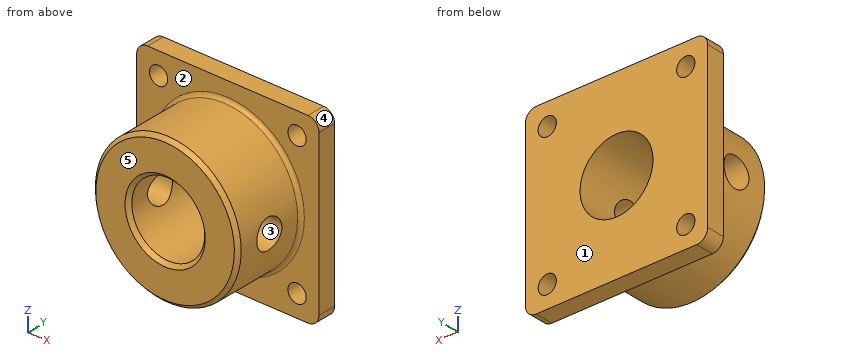
from build123d import *

# Parameters (mm, degrees)
SKETCH1_R               = 20
BOSS_EXTRUDE1_DEPTH     = 20
CUT_EXTRUDE5_DEPTH      = 25
CUT_EXTRUDE5_DEPTH_BACK = 25
SKETCH8_R               = 4
SKETCH9_W               = 50
SKETCH9_H               = 50
BOSS_EXTRUDE3_DEPTH     = 5
SKETCH10_R              = 10
CUT_EXTRUDE6_DEPTH      = 25
SKETCH11_R              = 2.5
CUT_EXTRUDE7_DEPTH      = 10
FILLET1_R               = 3
FILLET2_R               = 1
CHAMFER1_SIZE           = 1


with BuildPart() as part:
    # Sketch1 → Boss-Extrude1 (new body)
    with BuildSketch(Plane(origin=(0, 0, 0), x_dir=(1, 0, 0), z_dir=(0, 1, 0))):
        with Locations(Location((0, 0, 0), (0, 0, 270))):
            Circle(SKETCH1_R)
    extrude(amount=BOSS_EXTRUDE1_DEPTH)

    # Sketch8 → Cut-Extrude5 (cut, two sides: drawn at the far end of the back side and taken through both)
    with BuildSketch(Plane(origin=(0, 0, 0), x_dir=(0, 0, -1), z_dir=(1, 0, 0)).offset(-CUT_EXTRUDE5_DEPTH_BACK)):
        with Locations(Location((0, 10, 0), (0, 0, 180))):
            Circle(SKETCH8_R)
    extrude(amount=CUT_EXTRUDE5_DEPTH + CUT_EXTRUDE5_DEPTH_BACK, mode=Mode.SUBTRACT)

    # Sketch9 → Boss-Extrude3 (add)
    with BuildSketch(Plane(origin=(0, 20, 0), x_dir=(1, 0, 0), z_dir=(0, 1, 0))):
        Rectangle(SKETCH9_W, SKETCH9_H)
    extrude(amount=BOSS_EXTRUDE3_DEPTH)

    # Sketch10 → Cut-Extrude6 (cut)
    with BuildSketch(Plane(origin=(0, 25, 0), x_dir=(1, 0, 0), z_dir=(0, 1, 0))):
        with Locations(Location((0, 0, 0), (0, 0, 270))):
            Circle(SKETCH10_R)
    extrude(amount=-CUT_EXTRUDE6_DEPTH, mode=Mode.SUBTRACT)

    # Sketch11 → Cut-Extrude7 (cut)
    with BuildSketch(Plane(origin=(0, 25, 0), x_dir=(1, 0, 0), z_dir=(0, 1, 0))):
        with Locations(Location((-19, 19, 0), (0, 0, 270))):
            Circle(SKETCH11_R)
        with Locations(Location((-19, -19, 0), (0, 0, 270))):
            Circle(SKETCH11_R)
        with Locations(Location((19, -19, 0), (0, 0, 270))):
            Circle(SKETCH11_R)
        with Locations(Location((19, 19, 0), (0, 0, 270))):
            Circle(SKETCH11_R)
    extrude(amount=-CUT_EXTRUDE7_DEPTH, mode=Mode.SUBTRACT)

    # Fillet1
    fillet1_edges = [part.edges().sort_by_distance(p)[0] for p in [
        (25, 22.5, 25),
        (25, 22.5, -25),
        (-25, 22.5, -25),
        (-25, 22.5, 25),
    ]]
    fillet(fillet1_edges, radius=FILLET1_R)

    # Fillet2
    fillet2_edges = [part.edges().sort_by_distance(p)[0] for p in [
        (0, 20, -20),
    ]]
    fillet(fillet2_edges, radius=FILLET2_R)

    # Chamfer1
    chamfer1_edges = [part.edges().sort_by_distance(p)[0] for p in [
        (0, 0, -20),
        (0, 0, -10),
    ]]
    chamfer(chamfer1_edges, length=CHAMFER1_SIZE)


solid = part.part
Part model, mm, in its own coordinate system. Face numbers are marked on the shaded views. A direction names the side the tool comes from. Coordinates: 2 decimals unless noted, no trailing zeros. Order: outer loops, then holes, each group sorted by start corner. A loop starts at its lowest first (then second) coordinate and runs counter-clockwise, first axis right, second up. Notation, with made-up numbers: (0, 68) - (55, 68) arc R19 cw to (55, 93) - close; hole circle Ø10 at (-8.5, 50). An arc over 180 degrees is marked (long way). Use CSV: the item, a comma, the result in double quotes.
Item 1: Saw through at C-C on y = 16. Give the cut face in (x, z).
Solved:
outline,"circle Ø40 at (0, 0); hole circle Ø20 at (0, 0)"
Item 2: Mould opens along Y. For the marked faces 3, 4 and 5 say: +Y half, -Y half, draft (parallel to the pull), parting line (faces both ways), or undercut.
Solved:
face 3,"undercut"
face 4,"draft"
face 5,"-Y half"
Item 3: 3-axis set-ups, long thin cutter, end or side, ignore diameter. For the marked faces 1 and 2: which of +Z, -Z, +X, -X, +Y, -Y reach the whole face in a straight line?
Solved:
face 1,"+Z, -Z, +X, -X, +Y"
face 2,"-Y"
Item 4: Drop flat-ended pins along their axis: P1, Ø6.5, axis at x = 19, z = 19, coming from the -Y side; P2, Ø6, axis at y = 5, z = -0.5, coming from the -X side; P3, Ø10, axis at x = -19.5, y = 5.5, coming from the -Z side (3 decimals). Give the stop position or say it passes through.
Solved:
P1,"stops at y = 20"
P2,"stops at x = -20"
P3,"stops at z = -13.775"
Item 5: Probe probe 1 along X at (y, z) = (22.3, -19); probe 2 along Y at (x, z) = (12.5, 0); probe 3 along Y at (x, z) = (21, -3.5). List the from-to ranges inside material, lowest first.
Solved:
probe 1,"x = -25 to -21.5, -16.5 to 16.5, 21.5 to 25"
probe 2,"y = 0 to 6, 14 to 25"
probe 3,"y = 20 to 25"
Item 6: Saw through at B-B on y = 6.75. Give the cut face in (x, z).
Solved:
outline,"(-19.86, -2.33) arc R20 ccw to (19.86, -2.33) - (9.72, -2.33) arc R10 cw to (-9.72, -2.33) - close; (-19.86, 2.33) - (-9.72, 2.33) arc R10 cw to (9.72, 2.33) - (19.86, 2.33) arc R20 ccw to start"
Item 7: Saw through at D-D on y = 12. Give the cut face in (x, z).
Solved:
outline,"(-19.7, -3.46) arc R20 ccw to (19.7, -3.46) - (9.38, -3.46) arc R10 cw to (-9.38, -3.46) - close; (-19.7, 3.46) - (-9.38, 3.46) arc R10 cw to (9.38, 3.46) - (19.7, 3.46) arc R20 ccw to start"
Item 8: Saw through at A-A on z = 0. Give the cut face in (x, y).
Solved:
outline,"(-25, 20) - (-21, 20) arc R1 cw to (-20, 19) - (-20, 14) - (-10, 14) - (-10, 25) - (-25, 25) - close; (-20, 1) - (-19, 0) - (-11, 0) - (-10, 1) - (-10, 6) - (-20, 6) - close; (10, 1) - (11, 0) - (19, 0) - (20, 1) - (20, 6) - (10, 6) - close; (10, 14) - (20, 14) - (20, 19) arc R1 cw to (21, 20) - (25, 20) - (25, 25) - (10, 25) - close"
